Input: dimensioned drawing with shaded views. Units: mm. Origin: part minimum x, y, z. A direction names the side the tool comes from. Give positions to 0.01 mm unless a question says otherwise; leave off trailing zeros. Write each loop counter-clockwise with the first axis right and the second up, starting at its lowest first coordinate (ties: lowest second). Pieces come first, ordered by that corner, then holes. Notation, with made-up numbers: (53, 87.5) -> (80, 87.5) arc R31 cw to (80, 117.5) -> close; hole circle Ø3 at (-10.75, 74.5). An arc over 180 degrees is marked (long way). Return JSON: item names as keys, results as strings. Group by question number.
Item 1: Section B-B, the plane y = 10. Return loops of the section in (x, z).
Item 2: Line query: line 1 (Y direction, x = 4, z = 5); line 2 (Y direction, x = 6.5, z = 4); line 3 (Z direction, x = 0.5, y = 9.5). Output: solid intervals per line, ascending. Write a range as [from, to].
Item 3: Section C-C, the plane x = 4. Return loops of the section in (y, z).
Item 4: Section A-A, the plane z = 5. Return loops of the section in (x, y).
Item 5: Set-up query: the marked faces 5, 6 and 7. Return all of +Z, -Z, +X, -X, +Y, -Y with unobstructed straight access to the full face (end or side cutting, diameter ignored); none if empty.
Item 6: Section D-D, the plane y = 33. Return loops of the section in (x, z), then the cut area to 3 significant figures.
Item 7: Mould query, pull axis Z, two halves, no side actions, for the marked faces 1, 2, 3 and 4. Classes: released by +Z, released by -Z, zero draft, split by the parting line, or undercut.
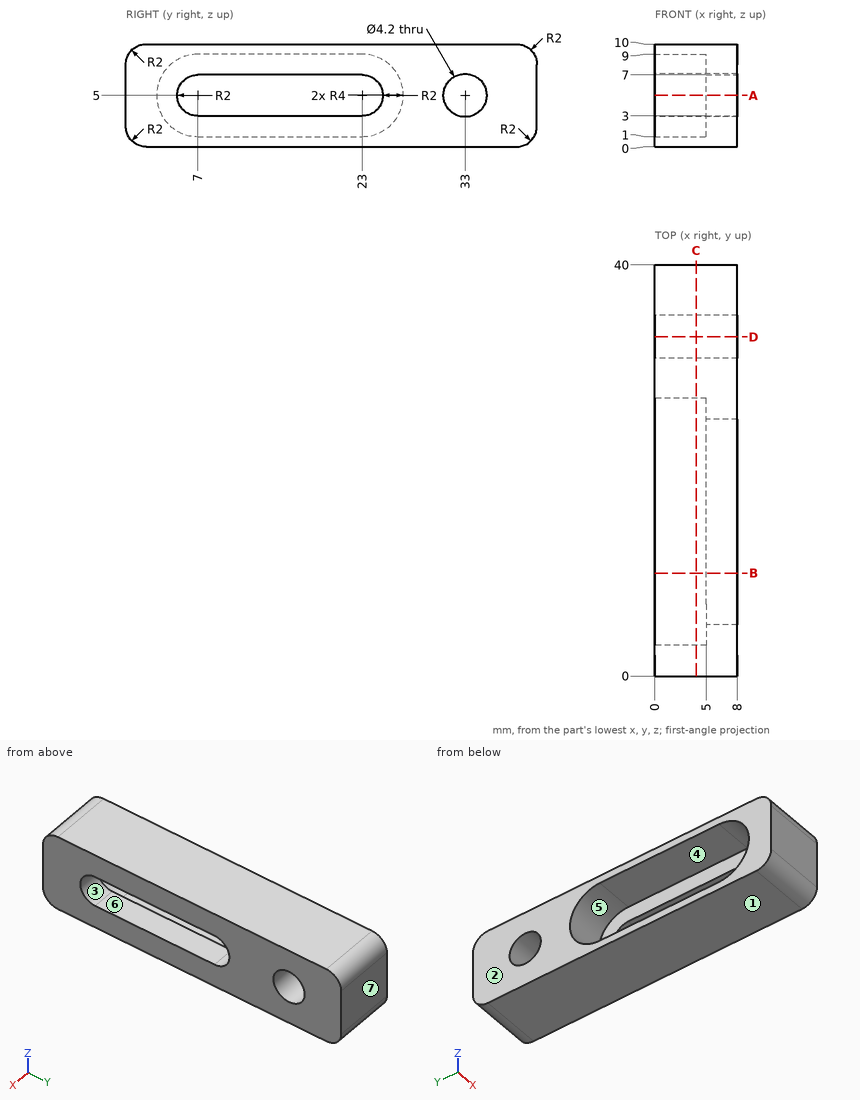
Answer below:
{
 "1": {"outline": "(0, 0) -> (8, 0) -> (8, 3) -> (5, 3) -> (5, 1) -> (0, 1) -> close; (0, 9) -> (5, 9) -> (5, 7) -> (8, 7) -> (8, 10) -> (0, 10) -> close"},
 "2": {"line 1": "y = [0, 3], [27, 30.9], [35.1, 40]", "line 2": "y = [0, 5.27], [24.73, 31.15], [34.85, 40]", "line 3": "z = [0, 1], [9, 10]"},
 "3": {"outline": "(0, 2) arc R2 ccw to (2, 0) -> (38, 0) arc R2 ccw to (40, 2) -> (40, 8) arc R2 ccw to (38, 10) -> (2, 10) arc R2 ccw to (0, 8) -> close; hole (7, 1) -> (23, 1) arc R4 ccw to (23, 9) -> (7, 9) arc R4 ccw to start; hole circle Ø4.2 at (33, 5)"},
 "4": {"outline": "(0, 0) -> (8, 0) -> (8, 5) -> (5, 5) -> (5, 3) -> (0, 3) -> close; (0, 27) -> (5, 27) -> (5, 25) -> (8, 25) -> (8, 30.9) -> (0, 30.9) -> close; (0, 35.1) -> (8, 35.1) -> (8, 40) -> (0, 40) -> close"},
 "5": {"face 5": "-X", "face 6": "+X, -X", "face 7": "+Z, -Z, +X, -X, +Y"},
 "6": {"outline": "(0, 0) -> (8, 0) -> (8, 2.9) -> (0, 2.9) -> close; (0, 7.1) -> (8, 7.1) -> (8, 10) -> (0, 10) -> close", "area": "46.4 mm2"},
 "7": {"face 1": "released by -Z", "face 2": "zero draft", "face 3": "undercut", "face 4": "undercut"}
}
